from build123d import *

# Parameters (mm, degrees)
BOSS_EXTRUDE1_DEPTH = 20
FILLET1_R           = 2
SKETCH2_R           = 7.5
BOSS_EXTRUDE2_DEPTH = 400
SKETCH3_W           = 40
SKETCH3_H           = 50
BOSS_EXTRUDE3_DEPTH = 10
SKETCH4_W           = 8.2
SKETCH4_H           = 50
BOSS_EXTRUDE4_DEPTH = 10


with BuildPart() as part:
    # Sketch1 → Boss-Extrude1 (new, symmetric)
    with BuildSketch(Plane.XY):
        Polygon((-10.5, 8), (-10.5, -8), (10.5, -8), (10.5, 8), (10.5, 15), (17.5, 15), (17.5, -15), (-17.5, -15), (-17.5, 15), (-10.5, 15), align=None)
    extrude(amount=BOSS_EXTRUDE1_DEPTH, both=True)

    # Fillet1
    fillet1_edges = [part.edges().sort_by_distance(p)[0] for p in [
        (17.5, -15, 0),
        (-17.5, -15, 0),
        (-10.5, -8, 0),
        (10.5, -8, 0),
    ]]
    fillet(fillet1_edges, radius=FILLET1_R)

    # Sketch2 → Boss-Extrude2 (add)
    with BuildSketch(Plane.XZ.offset(15)):
        with Locations(Location((0, 0, 0), (0, 0, 180))):
            Circle(SKETCH2_R)
    extrude(amount=BOSS_EXTRUDE2_DEPTH)

    # Sketch3 → Boss-Extrude3 (add)
    with BuildSketch(Plane.XZ.offset(415)):
        Rectangle(SKETCH3_W, SKETCH3_H)
    extrude(amount=BOSS_EXTRUDE3_DEPTH)

    # Sketch4 → Boss-Extrude4 (add)
    with BuildSketch(Plane.XZ.offset(425)):
        with Locations((-11, 0)):
            Rectangle(SKETCH4_W, SKETCH4_H)
        with Locations((11, 0)):
            Rectangle(SKETCH4_W, SKETCH4_H)
    extrude(amount=BOSS_EXTRUDE4_DEPTH)


solid = part.part
CAD build for the part. Positions are in the model's coordinates, mm. A direction names the side the tool comes from. Coordinates: 2 decimals unless noted, no trailing zeros. Order: outer loops, then holes, each group sorted by start corner. A loop starts at its lowest first (then second) coordinate and runs counter-clockwise, first axis right, second up.
Item 1: Band-saw the part on A-A on z = 11.5. List the corners of the cut face in (x, y), plus the area to 3 significant figures.
Check sheet entries:
outline: (-20, -425) - (-15.1, -425) - (-15.1, -435) - (-6.9, -435) - (-6.9, -425) - (6.9, -425) - (6.9, -435) - (15.1, -435) - (15.1, -425) - (20, -425) - (20, -415) - (-20, -415) - close; (-17.5, -13) arc R2 ccw to (-15.5, -15) - (15.5, -15) arc R2 ccw to (17.5, -13) - (17.5, 15) - (10.5, 15) - (10.5, -6) arc R2 cw to (8.5, -8) - (-8.5, -8) arc R2 cw to (-10.5, -6) - (-10.5, 15) - (-17.5, 15) - close
area: 1,130 mm2
Item 2: Band-saw the part on C-C on y = -129. List the corners of the cut face in (x, z).
Check sheet entries:
outline: circle Ø15 at (0, 0)
Item 3: 3-axis set-ups, long thin cutter, end or side, ignore diameter. For faces 4 (the face through (0, -8, 0)), 5 (the face through (15.1, -430, 0)), 6 (the face through (17.5, 1, 0)), 7 (the face through (0, -425, 0)), 8 (the face through (-5, -415, 6)): which of +Z, -Z, +X, -X, +Y, -Y reach the whole face in a straight line?
Check sheet entries:
face 4: +Z, -Z, +Y
face 5: +Z, -Z, +X, -Y
face 6: +Z, -Z, +X, +Y
face 7: +Z, -Z, -Y
face 8: none
Item 4: Two-plate mould, pull along X, no slides. Class faces 1 (the face through (10.5, 5, 0)), 2 (the face through (11, -435, 0)), 3 (the face through (-17.5, 1, 0)): +X half, -X half, draft (parallel to the pull), parting line (faces both ways), or undercut.
Check sheet entries:
face 1: undercut
face 2: draft
face 3: -X half
Item 5: Band-saw the part on B-B on x = 0. List the corners of the cut face in (y, z).
Check sheet entries:
outline: (-425, -25) - (-415, -25) - (-415, -7.5) - (-15, -7.5) - (-15, -20) - (-8, -20) - (-8, 20) - (-15, 20) - (-15, 7.5) - (-415, 7.5) - (-415, 25) - (-425, 25) - close
Item 6: Drill centre lines: L1, parallel to Y at x = -8.5, z = 19.5; L2, parallel to Z at x = 3, y = -79; L3, parallel to Z at x = 1, y = -85. Where is each one in solid material? Low to high.
Check sheet entries:
L1: y = -435 to -415, -15 to -8
L2: z = -6.87 to 6.87
L3: z = -7.43 to 7.43
Item 7: Pin check, flat tips, straight feed: pin 1 Ø22.5 at (y, z) = (5, 7.5) entering from -X; pin 2 Ø4 at (x, y) = (6, -321) entering from -Z; pin 3 Ø5.5 at (x, z) = (16.5, 4.5) entering from -Y; pin 4 Ø8 at (y, z) = (-431.5, 0.5) entering from -X. Stop position of each tip, or through.
Check sheet entries:
pin 1: stops at x = -17.5
pin 2: stops at z = -6.34
pin 3: stops at y = -435
pin 4: stops at x = -15.1
